Design review of the part built by this model. Coordinates are the model's own, in mm. Face numbers are marked on the shaded views. Coordinates: 2 decimals unless noted, no trailing zeros. Loops run counter-clockwise (first coordinate to the right, second up) from the corner with the lowest first, then second, coordinate; pieces in that order, holes last. Notation, with made-up numbers: (47, 51) - (88, 51) arc R24 cw to (88, 70) - close; hole circle Ø6 at (8.5, 85). An arc over 180 degrees is marked (long way). One line per question, with ' | ' between items.
from build123d import *

# Parameters (mm, degrees)
SKETCH_1_R          = 47.5
SKETCH_1_R_2        = 21
EXTRUDE_1_DEPTH     = 62
CHAMFER_1_SIZE      = 8
SKETCH_2_R          = 4
CUT_EXTRUDE_1_DEPTH = 92.413893911
M10X1_0_1_D         = 9
M10X1_0_1_DEPTH     = 10
M10X1_0_1_TIP       = 2.703872786


with BuildPart() as part:
    # 草图1 → 凸台-拉伸1 (new body)
    with BuildSketch(Plane.XY):
        Circle(SKETCH_1_R)
        Circle(SKETCH_1_R_2, mode=Mode.SUBTRACT)
    extrude(amount=EXTRUDE_1_DEPTH)

    # 倒角1
    chamfer_1_edges = [part.edges().sort_by_distance(p)[0] for p in [
        (-47.5, 0, 62),
    ]]
    chamfer(chamfer_1_edges, length=CHAMFER_1_SIZE)

    # 草图2 → 切除-拉伸1 (cut, through all)
    with BuildSketch(Plane(origin=(0, 0, 0), x_dir=(1, 0, 0), z_dir=(0, 1, 0))):
        with Locations(Location((0, -30, 0), (0, 0, 270))):
            Circle(SKETCH_2_R)
    extrude(amount=-CUT_EXTRUDE_1_DEPTH, mode=Mode.SUBTRACT)

    # M10x1.0 螺纹孔1
    with Locations(Plane.XZ.offset(47.5)):
        with Locations((0, 30)):
            Hole(M10X1_0_1_D / 2, depth=M10X1_0_1_DEPTH)
            with Locations((0, 0, -(M10X1_0_1_DEPTH + M10X1_0_1_TIP / 2))):  # 118° drill point
                Cone(0, M10X1_0_1_D / 2, M10X1_0_1_TIP, mode=Mode.SUBTRACT)


solid = part.part
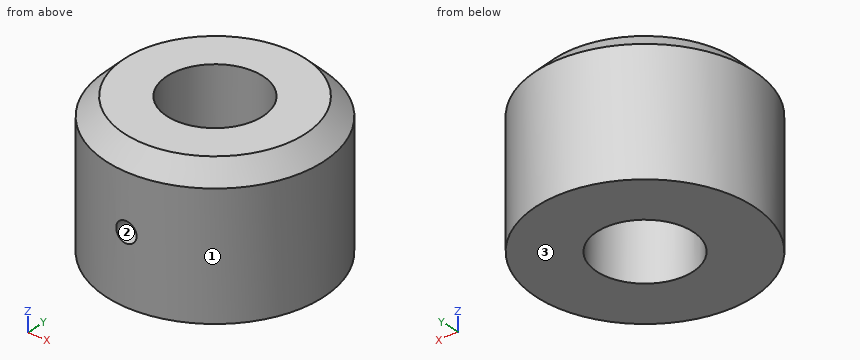
Q1. Take a section at C-C (z = 30). Give the boundary of the cut face in (x, y), plus the area to 3 significant figures.
Returned:
outline: (-4.5, -47.29) - (-4.5, -37.5) - (-4, -37.2) - (-4, -20.62) arc R21 cw (long way) to (4, -20.62) - (4, -37.2) - (4.5, -37.5) - (4.5, -47.29) arc R47.5 ccw (long way) to start | area: 5,480 mm²
Q2. For pin 1 (5 mm diameter, centred on y = 23, z = 42.5, fed in from -X); pin 2 (6.5 mm diameter, centred on x = 0, z = 30, fed in from -Y); pin 3 (1 mm diameter, centred on y = 16.5, z = 16, fed in from +X), all flat-tipped, find the tip position at first contact; note any pin that passes through.
Returned:
pin 1: stops at x = -42.85 | pin 2: stops at y = 20.75 | pin 3: stops at x = 44.72
Q3. To check wall thickness, follow line 1 along Z through (x, y) = (0, -25); line 2 along X through (y, z) = (-41.5, 31); line 3 along Y through (x, z) = (4, 21). State the ranges of each line that lie inside material, in increasing order.
Returned:
line 1: z = 0 to 26, 34 to 62 | line 2: x = -23.11 to -4.39, 4.39 to 23.11 | line 3: y = -47.33 to -20.62, 20.62 to 47.33
Q4. Draft analysis for pull direction X (two halves, no side actions). For the marked faces 1, 2 and 3, state which applies: +X half, -X half, draft (parallel to the pull), parting line (faces both ways), or undercut.
Returned:
face 1: parting line | face 2: undercut | face 3: draft
Q5. Take a section at B-B (y = 0). Give the boundary of the cut face in (x, z).
Returned:
outline: (-47.5, 0) - (-21, 0) - (-21, 62) - (-39.5, 62) - (-47.5, 54) - close; (21, 0) - (47.5, 0) - (47.5, 54) - (39.5, 62) - (21, 62) - close
Q6. Take a section at D-D (z = 45.5). Give the boundary of the cut face in (x, y).
Returned:
outline: circle Ø95 at (0, 0); hole circle Ø42 at (0, 0)
Q7. Take a section at A-A (x = 0). Give the boundary of the cut face in (y, z), plus the area to 3 significant figures.
Returned:
outline: (-47.5, 0) - (-21, 0) - (-21, 26) - (-37.2, 26) - (-37.5, 25.5) - (-47.5, 25.5) - close; (-47.5, 34.5) - (-37.5, 34.5) - (-37.2, 34) - (-21, 34) - (-21, 62) - (-39.5, 62) - (-47.5, 54) - close; (21, 0) - (47.5, 0) - (47.5, 54) - (39.5, 62) - (21, 62) - close | area: 3,000 mm²
